Read the model definition and answer for the solid it produces. Units are mm, in the model's axes. A direction names the side the tool comes from. Coordinates: 2 decimals unless noted, no trailing zeros. Write each loop counter-clockwise with the first axis right and the second up, starting at its lowest first coordinate (ties: lowest second). Pieces come first, ordered by that corner, then holes.
(1) Section A-A on x = -6.5 is taken. Write down the section's boundary in (y, z), then the cut area to 3 significant figures.
(2) Section B-B on z = 0 is taken. Write down the section's boundary in (x, y).
(3) Section C-C on y = 36.5 is taken. Write down the section's boundary in (x, z).
(4) Which of the six approach directions +Z, -Z, +X, -X, +Y, -Y give full straight-line access (tool end or side, diameter ignored) to faces 4 (the cylindrical face through (-99.99, 39.44, -0.88)), 5 (the flat face through (43, 7, 50)), 6 (the flat face through (95, 88, 25)), 7 (the flat face through (85, 68, -10))?
(5) Find the intervals of material crossed by probe 1 along Z at (x, y) = (45, 4.75); probe 2 along Y at (x, z) = (-6, -16); probe 3 along X at (y, z) = (90, -21.7), in increasing order.
(6) Section D-D on x = -54.5 is taken. Write down the section's boundary in (y, z).
(7) Given pin 1 (4 mm diameter, centred on x = -6, z = 28.5, fed in from +Y); pin 2 (8 mm diameter, centred on y = 18.5, z = -55.5, fed in from -X); pin 3 (8 mm diameter, centred on x = 45, z = -55, fed in from +Y); pin 4 (20 mm diameter, centred on x = 108, y = 83.5, fed in from -Z), each flat-ended and moving along its own axis, determine where each tip first touches the part or whether it passes through.
(8) The mould has two halves that part along Y. Classify faces 1 (the cylindrical face through (-8.67, 30.24, 0.56)), 2 (the flat face through (50, 47, 0)), 3 (the flat face through (-14, 80, 32)): +Y half, -Y half, draft (parallel to the pull), parting line (faces both ways), or undercut.
from build123d import *

# Parameters (mm, degrees)
BASE_PLATE_SKETCH_R       = 5
BASE_PLATE_DEPTH          = 15
HOUSING_WALL_DEPTH        = 65
EAR_RECESSES_SKETCH_R     = 10
EAR_RECESSES_2X_20_DEPTH  = 8
CROSS_BORE_SKETCH_R       = 10
CROSS_BORE_DEPTH          = 120
CROSS_START               = 60
CROSS_PIN_SKETCH_R        = 20
CROSS_PIN_SKETCH_R_2      = 10
CROSS_PIN_DEPTH           = 60
LUG_1_SKETCH_R            = 20
LUG_1_SKETCH_R_2          = 10
LUG_1_DEPTH               = 10
LUG_1_PIN_BOSS_SKETCH_R   = 20
LUG_1_PIN_BOSS_SKETCH_R_2 = 10
LUG_1_PIN_BOSS_DEPTH      = 5
LUG_START                 = -10
LUG_2_SKETCH_R            = 20
LUG_2_SKETCH_R_2          = 10
LUG_2_DEPTH               = 10
LUG_START_2               = 5
LUG_2_PIN_BOSS_SKETCH_R   = 20
LUG_2_PIN_BOSS_SKETCH_R_2 = 10
LUG_2_PIN_BOSS_DEPTH      = 5


with BuildPart() as part:
    # Base Plate Sketch → Base Plate (new body)
    # profile 1 of 3: a face of its own
    with BuildSketch(Plane(origin=(0, 0, 0), x_dir=(1, 0, 0), z_dir=(0, 1, 0))):
        with BuildLine():
            Line((-60, -40), (45, -40))
            ThreePointArc((45, -40), (55.606601718, -35.606601718), (60, -25))
            Line((60, -25), (60, 25))
            ThreePointArc((60, 25), (55.606601718, 35.606601718), (45, 40))
            Line((45, 40), (-60, 40))
            ThreePointArc((-60, 40), (-100, 0), (-60, -40))
        make_face()
    # profile 2 of 3: a face of its own
    with BuildSketch(Plane(origin=(0, 0, 0), x_dir=(1, 0, 0), z_dir=(0, 1, 0))):
        with BuildLine():
            Line((60, -40), (60, -25))
            ThreePointArc((60, -25), (55.606601718, -35.606601718), (45, -40))
            Line((45, -40), (5, -40))
            Line((5, -40), (33.441882385, -64.560853371))
            Line((33.441882385, -64.560853371), (37.224740847, -67.827522953))
            ThreePointArc((37.224740847, -67.827522953), (52.361083912, -68.06959998), (60, -55))
            Line((60, -55), (60, -40))
        make_face()
        with Locations(Location((45, -55, 0), (0, 0, 270))):
            Circle(BASE_PLATE_SKETCH_R, mode=Mode.SUBTRACT)
    # profile 3 of 3: a face of its own
    with BuildSketch(Plane(origin=(0, 0, 0), x_dir=(1, 0, 0), z_dir=(0, 1, 0))):
        with BuildLine():
            Line((60, 40), (60, 55))
            ThreePointArc((60, 55), (52.361083912, 68.06959998), (37.224740847, 67.827522953))
            Line((37.224740847, 67.827522953), (33.441882385, 64.560853371))
            Line((33.441882385, 64.560853371), (5, 40))
            Line((5, 40), (45, 40))
            ThreePointArc((45, 40), (55.606601718, 35.606601718), (60, 25))
            Line((60, 25), (60, 40))
        make_face()
        with Locations(Location((45, 55, 0), (0, 0, 270))):
            Circle(BASE_PLATE_SKETCH_R, mode=Mode.SUBTRACT)
    extrude(amount=BASE_PLATE_DEPTH)

    # Housing Wall Sketch → Housing Wall (add)
    with BuildSketch(Plane(origin=(0, 15, 0), x_dir=(1, 0, 0), z_dir=(0, 1, 0))):
        with BuildLine():
            Line((45, 40), (-60, 40))
            ThreePointArc((-60, 40), (-100, 0), (-60, -40))
            Line((-60, -40), (45, -40))
            ThreePointArc((45, -40), (55.606601718, -35.606601718), (60, -25))
            Line((60, -25), (60, 25))
            ThreePointArc((60, 25), (55.606601718, 35.606601718), (45, 40))
        make_face()
        with BuildLine():
            Line((45, 30), (-60, 30))
            ThreePointArc((-60, 30), (-90, 0), (-60, -30))
            Line((-60, -30), (45, -30))
            ThreePointArc((45, -30), (48.535533906, -28.535533906), (50, -25))
            Line((50, -25), (50, 25))
            ThreePointArc((50, 25), (48.535533906, 28.535533906), (45, 30))
        make_face(mode=Mode.SUBTRACT)
    extrude(amount=HOUSING_WALL_DEPTH)

    # Ear Recesses Sketch → Ear Recesses 2xØ20 (cut)
    with BuildSketch(Plane(origin=(0, 15, 0), x_dir=(1, 0, 0), z_dir=(0, 1, 0))):
        with Locations(Location((45, -55, 0), (0, 0, 270))):
            Circle(EAR_RECESSES_SKETCH_R)
        with Locations(Location((45, 55, 0), (0, 0, 270))):
            Circle(EAR_RECESSES_SKETCH_R)
    extrude(amount=-EAR_RECESSES_2X_20_DEPTH, mode=Mode.SUBTRACT)

    # Cross Bore Sketch → Cross Bore (cut)
    with BuildSketch(Plane.XY.offset(40)):
        with Locations((-6.5, 40)):
            Circle(CROSS_BORE_SKETCH_R)
    extrude(amount=-CROSS_BORE_DEPTH, mode=Mode.SUBTRACT)

    # Cross Pin Sketch → Cross Pin (add)
    with BuildSketch(Plane.XY.offset(-30).offset(CROSS_START)):
        with Locations((-6.5, 40)):
            Circle(CROSS_PIN_SKETCH_R)
        with Locations((-6.5, 40)):
            Circle(CROSS_PIN_SKETCH_R_2, mode=Mode.SUBTRACT)
    extrude(amount=-CROSS_PIN_DEPTH)

    # Lug 1 Sketch → Lug 1 (add)
    # profile 1 of 2: a face of its own
    with BuildSketch(Plane.XY.offset(10)):
        with BuildLine():
            Line((92.6204123, 105.708144651), (60, 80))
            Line((60, 80), (60, 0))
            Line((60, 0), (120.753851487, 77.678629812))
            ThreePointArc((120.753851487, 77.678629812), (90.884057256, 75.831719919), (92.6204123, 105.708144651))
        make_face()
    # profile 2 of 2: a face of its own
    with BuildSketch(Plane.XY.offset(10)):
        with Locations((105, 90)):
            Circle(LUG_1_SKETCH_R)
        with Locations((105, 90)):
            Circle(LUG_1_SKETCH_R_2, mode=Mode.SUBTRACT)
    extrude(amount=LUG_1_DEPTH)

    # Lug 1 Pin Boss Sketch → Lug 1 Pin Boss (add)
    with BuildSketch(Plane.XY.offset(20)):
        with Locations(Location((105, 90, 0), (0, 0, 128.241642007))):
            Circle(LUG_1_PIN_BOSS_SKETCH_R)
        with Locations((105, 90)):
            Circle(LUG_1_PIN_BOSS_SKETCH_R_2, mode=Mode.SUBTRACT)
    extrude(amount=LUG_1_PIN_BOSS_DEPTH)

    # Lug 2 Sketch → Lug 2 (add)
    # profile 1 of 2: a face of its own
    with BuildSketch(Plane.XY.offset(-10).offset(LUG_START)):
        with BuildLine():
            ThreePointArc((120.753851487, 77.678629812), (90.884057256, 75.831719919), (92.6204123, 105.708144651))
            Line((92.6204123, 105.708144651), (60, 80))
            Line((60, 80), (60, 0))
            Line((60, 0), (120.753851487, 77.678629812))
        make_face()
    # profile 2 of 2: a face of its own
    with BuildSketch(Plane.XY.offset(-10).offset(LUG_START)):
        with Locations(Location((105, 90, 0), (0, 0, 128.241642007))):
            Circle(LUG_2_SKETCH_R)
        with Locations((105, 90)):
            Circle(LUG_2_SKETCH_R_2, mode=Mode.SUBTRACT)
    extrude(amount=LUG_2_DEPTH)

    # Lug 2 Pin Boss Sketch → Lug 2 Pin Boss (add)
    with BuildSketch(Plane(origin=(0, 0, -20), x_dir=(-1, 0, 0), z_dir=(0, 0, -1)).offset(LUG_START_2)):
        with Locations(Location((-105, 90, 0), (0, 0, 51.758357993))):
            Circle(LUG_2_PIN_BOSS_SKETCH_R)
        with Locations(Location((-105, 90, 0), (0, 0, 180))):
            Circle(LUG_2_PIN_BOSS_SKETCH_R_2, mode=Mode.SUBTRACT)
    extrude(amount=-LUG_2_PIN_BOSS_DEPTH)


solid = part.part
Response:
1. outline: (0, -40) - (30, -40) - (30, 40) - (0, 40) - close; (50, -40) - (80, -40) - (80, -30) - (60, -30) - (60, 30) - (80, 30) - (80, 40) - (50, 40) - close; hole (15, -30) - (20, -30) - (20, 30) - (15, 30) - close
1. area: 3,300 mm2
2. outline: (-100, 0) - (60, 0) - (60, 80) - (50, 80) - (50, 15) - (-90, 15) - (-90, 80) - (-100, 80) - close; circle Ø40 at (-6.5, 40); hole circle Ø20 at (-6.5, 40)
3. outline: (-60, -40) - (-15.87, -40) - (-15.87, 40) - (-60, 40) arc R40 ccw to start; (2.87, -40) - (45, -40) arc R15 ccw to (60, -25) - (60, -20) - (88.55, -20) - (88.55, -10) - (60, -10) - (60, 10) - (88.55, 10) - (88.55, 20) - (60, 20) - (60, 25) arc R15 ccw to (45, 40) - (2.87, 40) - close; hole (-60, -30) - (-26.19, -30) - (-26.19, 30) - (-60, 30) arc R30 ccw to start; hole (13.19, -30) - (45, -30) arc R5 ccw to (50, -25) - (50, 25) arc R5 ccw to (45, 30) - (13.19, 30) - close
4. face 4: -X, +Y, -Y
4. face 5: +Y
4. face 6: +Z, +X, +Y, -Y
4. face 7: +X, +Y, -Y
5. probe 1: z = -70 to -60, -50 to 50, 60 to 70
5. probe 2: y = 0 to 15, 20.01 to 30.01, 49.99 to 59.99
5. probe 3: x = 85 to 95, 115 to 125
6. outline: (0, -40) - (80, -40) - (80, -30) - (15, -30) - (15, 30) - (80, 30) - (80, 40) - (0, 40) - close
7. pin 1: stops at y = 80
7. pin 2: stops at x = 20.71
7. pin 3: passes through
7. pin 4: stops at z = -25
8. face 1: undercut
8. face 2: draft
8. face 3: +Y half
